Can you work these out from the model? Positions are in its coordinate system, mm. A direction names the side the tool comes from. Give positions to 0.01 mm unless a question says otherwise; leave off trailing zeros. Order: outer loops, then holes, each group sorted by start corner. A loop starts at its lowest first (then second) coordinate and runs counter-clockwise, first axis right, second up. Notation, with made-up numbers: (11, -30) - (19, -30) arc R14 cw to (19, -15) - close; hole circle Ø11 at (33, -16.75). An arc over 180 degrees is marked (long way). Answer as a JSON object with one key per item and string values.
```python
from build123d import *

# Parameters (mm, degrees)
SKETCH_1_R          = 35
EXTRUDE_1_DEPTH     = 15
SKETCH_2_R          = 25
EXTRUDE_2_DEPTH     = 35
EXTRUDE_START       = 35
SKETCH_3_R          = 25
EXTRUDE_3_DEPTH     = 35
CUT_EXTRUDE_1_DEPTH = 25
SKETCH_5_R          = 12.5
CUT_EXTRUDE_2_DEPTH = 25
CUT_EXTRUDE_3_DEPTH = 15


with BuildPart() as part:
    # 草图1 → 凸台-拉伸1 (new, symmetric)
    with BuildSketch(Plane.XY):
        Circle(SKETCH_1_R)
    extrude(amount=EXTRUDE_1_DEPTH, both=True)

    # 草图2 → 凸台-拉伸2 (add)
    with BuildSketch(Plane.XY.offset(15)):
        Circle(SKETCH_2_R)
    extrude(amount=EXTRUDE_2_DEPTH)

    # 草图3 → 凸台-拉伸3 (add)
    with BuildSketch(Plane(origin=(0, 0, -15), x_dir=(-1, 0, 0), z_dir=(0, 0, -1)).offset(EXTRUDE_START)):
        with Locations(Location((0, 0, 0), (0, 0, 180))):
            Circle(SKETCH_3_R)
    extrude(amount=-EXTRUDE_3_DEPTH)

    # 草图4 → 切除-拉伸1 (cut, symmetric)
    with BuildSketch(Plane.XY.offset(50)):
        with BuildLine():
            Line((-5.385, 17.5), (5.385, 17.5))
            Line((5.385, 17.5), (5.385, 12.651651078))
            ThreePointArc((5.385, 12.651651078), (0, -13.75), (-5.385, 12.651651078))
            Line((-5.385, 12.651651078), (-5.385, 17.5))
        make_face()
    extrude(amount=CUT_EXTRUDE_1_DEPTH, both=True, mode=Mode.SUBTRACT)

    # 草图5 → 切除-拉伸2 (cut, symmetric)
    with BuildSketch(Plane(origin=(0, 0, -50), x_dir=(-1, 0, 0), z_dir=(0, 0, -1))):
        Circle(SKETCH_5_R)
    extrude(amount=CUT_EXTRUDE_2_DEPTH, both=True, mode=Mode.SUBTRACT)

    # 草图6 → 切除-拉伸3 (cut, symmetric)
    with BuildSketch(Plane(origin=(0, 0, -50), x_dir=(-1, 0, 0), z_dir=(0, 0, -1))):
        with BuildLine():
            Line((-5, 15), (5, 15))
            Line((5, 15), (5, 11.456439237))
            ThreePointArc((5, 11.456439237), (0, 12.5), (-5, 11.456439237))
            Line((-5, 11.456439237), (-5, 15))
        make_face()
    extrude(amount=CUT_EXTRUDE_3_DEPTH, both=True, mode=Mode.SUBTRACT)


solid = part.part
```
Q1. We'd pull the mould along Y, two halves only. Please class faces 1 (the face through (-28, -21, 0)), 2 (the face through (-24, 8, -15)), 3 (the face through (-5, 13, -43)): released by +Y, released by -Y, zero draft, split by the parting line, or undercut.
Recorded:
{"face 1": "split by the parting line", "face 2": "zero draft", "face 3": "undercut"}
Q2. If we section it at D-D, the plane x = 21: Please give me the cut outline in (y, z), then the cut area to 3 significant figures.
Recorded:
{"outline": "(-28, -15) - (-13.56, -15) - (-13.56, -50) - (13.56, -50) - (13.56, -15) - (28, -15) - (28, 15) - (13.56, 15) - (13.56, 50) - (-13.56, 50) - (-13.56, 15) - (-28, 15) - close", "area": "3,580 mm^2"}
Q3. I need wall thicknesses on L1, parallel to Y at x = 0, z = 36.75; L2, parallel to X at y = 1, z = 24.5; L3, parallel to Z at x = 13, y = 30. Which ranges of each line are inside material? Lowest first, please.
Recorded:
{"L1": "y = -25 to -13.75, 17.5 to 25", "L2": "x = -24.98 to 24.98", "L3": "z = -15 to 15"}
Q4. If we section it at C-C, the plane x = 0: Please give me the cut outline in (y, z).
Recorded:
{"outline": "(-35, -15) - (-25, -15) - (-25, -50) - (-12.5, -50) - (-12.5, -25) - (12.5, -25) - (12.5, -35) - (15, -35) - (15, -50) - (25, -50) - (25, -15) - (35, -15) - (35, 15) - (25, 15) - (25, 50) - (17.5, 50) - (17.5, 25) - (-13.75, 25) - (-13.75, 50) - (-25, 50) - (-25, 15) - (-35, 15) - close"}
Q5. Which directions (+Z, -Z, +X, -X, +Y, -Y) give clear straight access to the entire face, cutting with the end or side of a thin tool? Please do faces 4 (the face through (0, 2, 25)), 5 (the face through (0, 0, -25)), 6 (the face through (-5.9, -11.5, -50)).
Recorded:
{"face 4": "+Z", "face 5": "-Z", "face 6": "-Z, +X, -X, +Y, -Y"}
Q6. If we section it at A-A, the plane z = 33: Please give me the cut outline in (x, y) (3 decimals).
Recorded:
{"outline": "circle Ø50 at (0, 0); hole (-5.385, 12.652) arc R13.75 ccw (long way) to (5.385, 12.652) - (5.385, 17.5) - (-5.385, 17.5) - close"}
Q7. I'm going to push flat-ended pins straight in: pin 1 Ø16.5 at (x, y) = (0, 0) entering from -Z; pin 2 Ø2 at (y, z) = (-9, 15) entering from +X; pin 3 Ø5 at (y, z) = (5, 38.5) entering from -X. Where does each tip first touch, or does it pass through?
Recorded:
{"pin 1": "stops at z = -25", "pin 2": "stops at x = 34.07", "pin 3": "stops at x = -24.87"}
Q8. If we section it at B-B, the plane y = 0: Please give me the cut outline in (x, z).
Recorded:
{"outline": "(-35, -15) - (-25, -15) - (-25, -50) - (-12.5, -50) - (-12.5, -25) - (12.5, -25) - (12.5, -50) - (25, -50) - (25, -15) - (35, -15) - (35, 15) - (25, 15) - (25, 50) - (13.75, 50) - (13.75, 25) - (-13.75, 25) - (-13.75, 50) - (-25, 50) - (-25, 15) - (-35, 15) - close"}
